Design review of the part built by this model. Coordinates are the model's own, in mm. Coordinates: 2 decimals unless noted, no trailing zeros. Write each loop counter-clockwise with the first axis right and the second up, starting at its lowest first coordinate (ties: lowest second). Pieces come first, ordered by that corner, then holes. Notation, with made-up numbers: (-1.5, -25.75) - (18.5, -25.75) arc R9 cw to (18.5, -14.75) - close; hole circle Ø10 at (76, 1.25). An arc over 180 degrees is marked (long way). One line per item, written item: value.
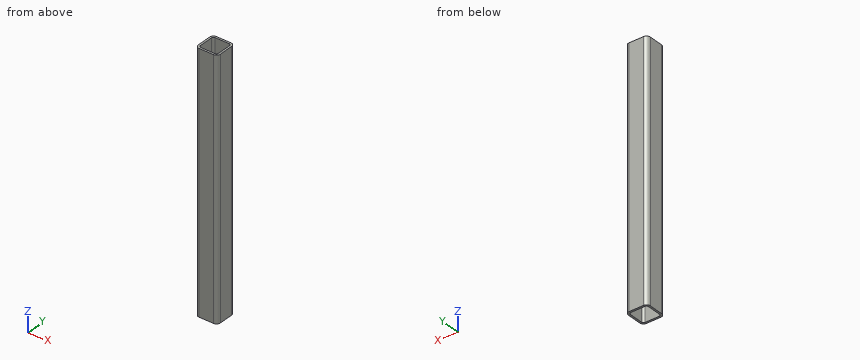
from build123d import *

# Parameters (mm, degrees)
BOSS_EXTRUDE1_DEPTH = 805


with BuildPart() as part:
    # Sketch1 → Boss-Extrude1 (new body)
    with BuildSketch(Plane.XY):
        with BuildLine():
            Line((12, 0), (58, 0))
            ThreePointArc((58, 0), (66.485281374, 3.514718626), (70, 12))
            Line((70, 12), (70, 58))
            ThreePointArc((70, 58), (66.485281374, 66.485281374), (58, 70))
            Line((58, 70), (12, 70))
            ThreePointArc((12, 70), (3.514718626, 66.485281374), (0, 58))
            Line((0, 58), (0, 12))
            ThreePointArc((0, 12), (3.514718626, 3.514718626), (12, 0))
        make_face()
        with BuildLine():
            Line((12, 6), (58, 6))
            ThreePointArc((58, 6), (62.242640687, 7.757359313), (64, 12))
            Line((64, 12), (64, 58))
            ThreePointArc((64, 58), (62.242640687, 62.242640687), (58, 64))
            Line((58, 64), (12, 64))
            ThreePointArc((12, 64), (7.757359313, 62.242640687), (6, 58))
            Line((6, 58), (6, 12))
            ThreePointArc((6, 12), (7.757359313, 7.757359313), (12, 6))
        make_face(mode=Mode.SUBTRACT)
    extrude(amount=BOSS_EXTRUDE1_DEPTH)


solid = part.part
1. Consider section A-A, the plane y = 51.5. Write out the cut boundary in (x, z), then the cut area to 3 significant figures.
Answer block:
outline: (0, 0) - (6, 0) - (6, 805) - (0, 805) - close; (64, 0) - (70, 0) - (70, 805) - (64, 805) - close
area: 9,660 mm^2
2. Wall thickness on line 1 along X through (y, z) = (35.5, 759.5); line 2 along Y through (x, z) = (9, 45): over which ranges is each line inside the solid? List them lowest first.
Answer block:
line 1: x = 0 to 6, 64 to 70
line 2: y = 0.38 to 6.8, 63.2 to 69.62
3. Consider section B-B, the plane z = 663.5. Write out the cut boundary in (x, y).
Answer block:
outline: (0, 12) arc R12 ccw to (12, 0) - (58, 0) arc R12 ccw to (70, 12) - (70, 58) arc R12 ccw to (58, 70) - (12, 70) arc R12 ccw to (0, 58) - close; hole (6, 12) arc R6 ccw to (12, 6) - (58, 6) arc R6 ccw to (64, 12) - (64, 58) arc R6 ccw to (58, 64) - (12, 64) arc R6 ccw to (6, 58) - close
